Work out the finished part from the listing and answer in its coordinate system (mm). Face numbers are marked on the shaded views. A direction names the side the tool comes from. Round coordinates to 2 decimals unless told otherwise and drop trailing zeros. Loops run counter-clockwise (first coordinate to the right, second up) from the corner with the lowest first, then second, coordinate; pieces in that order, holes last.
```python
from build123d import *

# Parameters (mm, degrees)
SKETCH1_W             = 100
SKETCH1_H             = 48
BOSS_EXTRUDE1_DEPTH   = 8
SKETCH2_W             = 46
SKETCH2_H             = 48
BOSS_EXTRUDE2_DEPTH   = 10
CUT_EXTRUDE1_DEPTH    = 72.61005516
FILLET1_R             = 8
M4_TAPPED_HOLE1_D     = 3.3
M4_TAPPED_HOLE1_DEPTH = 10
M4_TAPPED_HOLE1_TIP   = 0.991420021
M8_TAPPED_HOLE1_D     = 6.8


with BuildPart() as part:
    # Sketch1 → Boss-Extrude1 (new body)
    with BuildSketch(Plane(origin=(0, 0, 0), x_dir=(1, 0, 0), z_dir=(0, 1, 0))):
        Rectangle(SKETCH1_W, SKETCH1_H)
    extrude(amount=BOSS_EXTRUDE1_DEPTH)

    # Sketch2 → Boss-Extrude2 (add)
    with BuildSketch(Plane(origin=(0, 8, 0), x_dir=(1, 0, 0), z_dir=(0, 1, 0))):
        Rectangle(SKETCH2_W, SKETCH2_H)
    extrude(amount=BOSS_EXTRUDE2_DEPTH)

    # Sketch3 → Cut-Extrude1 (cut, through all)
    with BuildSketch(Plane.XY.offset(24)):
        with BuildLine():
            Line((-8, 13), (-8, 18))
            Line((-8, 18), (8, 18))
            Line((8, 18), (8, 13))
            ThreePointArc((8, 13), (0, 5), (-8, 13))
        make_face()
    extrude(amount=-CUT_EXTRUDE1_DEPTH, mode=Mode.SUBTRACT)

    # Fillet1
    fillet1_edges = [part.edges().sort_by_distance(p)[0] for p in [
        (50, 4, 24),
        (-50, 4, 24),
        (-50, 4, -24),
        (50, 4, -24),
    ]]
    fillet(fillet1_edges, radius=FILLET1_R)

    # M4 Tapped Hole1
    with Locations(Plane(origin=(0, 18, 0), x_dir=(1, 0, 0), z_dir=(0, 1, 0))):
        with Locations((-15, 14), (-15, -14), (15, -14), (15, 14)):
            Hole(M4_TAPPED_HOLE1_D / 2, depth=M4_TAPPED_HOLE1_DEPTH)
            with Locations((0, 0, -(M4_TAPPED_HOLE1_DEPTH + M4_TAPPED_HOLE1_TIP / 2))):  # 118° drill point
                Cone(0, M4_TAPPED_HOLE1_D / 2, M4_TAPPED_HOLE1_TIP, mode=Mode.SUBTRACT)

    # M8 Tapped Hole1 (through all)
    with Locations(Plane(origin=(0, 8, 0), x_dir=(1, 0, 0), z_dir=(0, 1, 0))):
        with Locations((-38, 12), (-38, -12), (38, -12), (38, 12)):
            Hole(M8_TAPPED_HOLE1_D / 2)


solid = part.part
```
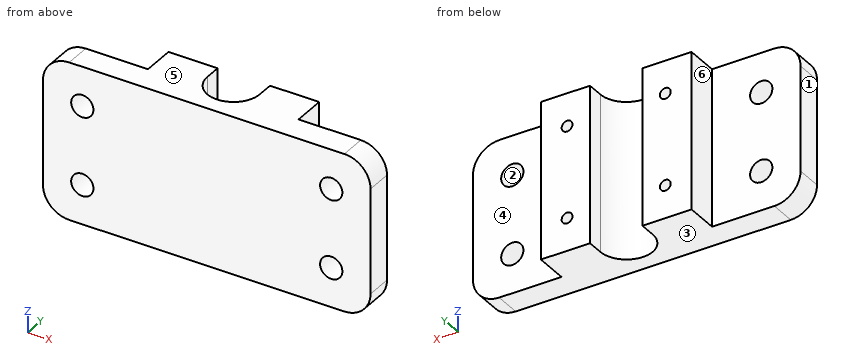
1. Given pin 1 (4 mm diameter, centred on y = 11.5, z = -2, fed in from +X); pin 2 (13.5 mm diameter, centred on x = -43, z = 6, fed in from +Y); pin 3 (1.5 mm diameter, centred on x = 4.5, z = 0.5, fed in from +Y), each flat-ended and moving along its own axis, determine where each tip first touches the part or whether it passes through.
Answer key:
pin 1: stops at x = 23
pin 2: stops at y = 8
pin 3: stops at y = 6.96
2. Find section A-A (y = 9.5). Write down the section's boundary in (x, z).
Answer key:
outline: (-23, -24) - (-7.19, -24) - (-7.19, 24) - (-23, 24) - close; (7.19, -24) - (23, -24) - (23, 24) - (7.19, 24) - close; hole circle Ø3.3 at (-15, -14); hole circle Ø3.3 at (-15, 14); hole circle Ø3.3 at (15, -14); hole circle Ø3.3 at (15, 14)
3. Consider probe 1 along X at (y, z) = (13.75, 14); probe 2 along Z at (x, y) = (-38, 2.25); probe 3 along X at (y, z) = (13.5, 7.5). Determine where each line is inside the solid, lowest interval first.
Answer key:
probe 1: x = -23 to -16.65, -13.35 to -8, 8 to 13.35, 16.65 to 23
probe 2: z = -24 to -15.4, -8.6 to 8.6, 15.4 to 24
probe 3: x = -23 to -8, 8 to 23
4. Find section B-B (x = -38). Write down the section's boundary in (y, z).
Answer key:
outline: (0, -24) - (8, -24) - (8, -15.4) - (0, -15.4) - close; (0, -8.6) - (8, -8.6) - (8, 8.6) - (0, 8.6) - close; (0, 15.4) - (8, 15.4) - (8, 24) - (0, 24) - close
5. Find section D-D (y = 2.75). Write down the section's boundary in (x, z).
Answer key:
outline: (-50, -16) arc R8 ccw to (-42, -24) - (42, -24) arc R8 ccw to (50, -16) - (50, 16) arc R8 ccw to (42, 24) - (-42, 24) arc R8 ccw to (-50, 16) - close; hole circle Ø6.8 at (-38, -12); hole circle Ø6.8 at (-38, 12); hole circle Ø6.8 at (38, -12); hole circle Ø6.8 at (38, 12)
6. Find section C-C (z = -6). Write down the section's boundary in (x, y).
Answer key:
outline: (-50, 0) - (50, 0) - (50, 8) - (23, 8) - (23, 18) - (8, 18) - (8, 13) arc R8 cw to (-8, 13) - (-8, 18) - (-23, 18) - (-23, 8) - (-50, 8) - close
7. Determine the mould class of the marked faces 1, 2 and 3 for opening direction Z: +Z half, -Z half, draft (parallel to the pull), parting line (faces both ways), or undercut.
Answer key:
face 1: draft
face 2: undercut
face 3: -Z half
8. Which of the six approach directions +Z, -Z, +X, -X, +Y, -Y give full straight-line access (tool end or side, diameter ignored) to the marked faces 4, 5 and 6?
Answer key:
face 4: +Z, -Z, +X, +Y
face 5: +Z, +X, -X, +Y, -Y
face 6: +Z, -Z, -X, +Y
